Could you check a few things on this model? Use its own coordinates, in mm. A direction names the side the tool comes from. Give positions to 0.01 mm unless a question says otherwise; leave off trailing zeros. Order: outer loops, then holes, each group sorted by start corner. A loop starts at its lowest first (then second) coordinate and runs counter-clockwise, first axis right, second up. Notation, with made-up numbers: M -34,13.5 L 17,13.5 A14 cw 17,26.5 Z; hole C 51.5,-27 d10. An arc over 180 degrees is marked long. Use a Markdown table: item, result. Add a question column.
Item 1: If I drill on L1, parallel to Y at x = 0, z = 54.5; L2, parallel to Y at x = 0, z = 62.5; L3, parallel to Z at x = -3.5, y = 6.25, over which ranges is the centre line in solid material (lowest first)? Write a range as from..to.
Item 2: Suppose I cut it at A-A on y = 0. Write out the boundary of the cut face in (x, z).
Item 3: For faces 1 (the face through (-3, -1, 125)), 2 (the face through (-6, 0, 90)), 3 (the face through (0, 7, 45)), which set-ups out of +Z, -Z, +X, -X, +Y, -Y let a thin tool reach every point of the face, with its end or its side?
Item 4: I'm going to push flat-ended pins straight in: pin 1 Ø5 at (y, z) = (3.5, 19.5) entering from -X; pin 2 Ø8 at (x, z) = (5, 21) entering from -Y; pin 3 Ø2 at (y, z) = (-5.5, 22.5) entering from +X; pin 4 Ø3.5 at (x, y) = (0, 0) entering from -Z. Where does each tip first touch, or does it pass through?
Item 5: Suppose I cut it at C-C on z = 103.5. Write out the boundary of the cut face in (x, y), plus the area to 3 significant figures.
Item 6: Suppose I cut it at D-D on z = 16. Write out the boundary of the cut face in (x, y), plus the area to 3 significant figures.
Item 7: If we mould it in two halves opening along X, with no side actions, what happens to faces 4 (the face through (-5.158, -3.955, 39.93)), 5 (the face through (1, 3, 0)), 6 (the face through (-3, 0, 62))? For each: released by +X, released by -X, zero draft, split by the parting line, or undercut.
from build123d import *

# Parameters (mm, degrees)
SKETCH1_R           = 5
SKETCH1_R_2         = 3
BOSS_EXTRUDE1_DEPTH = 35
SKETCH2_R           = 6.5
SKETCH2_R_2         = 3
BOSS_EXTRUDE2_DEPTH = 10
SKETCH3_R           = 8
SKETCH3_R_2         = 3
BOSS_EXTRUDE3_DEPTH = 10
SKETCH4_R           = 6
SKETCH4_R_2         = 3
BOSS_EXTRUDE4_DEPTH = 70
CHAMFER1_SIZE       = 1
CHAMFER1_SIZE2      = 10


with BuildPart() as part:
    # Sketch1 → Boss-Extrude1 (new body)
    with BuildSketch(Plane.XY):
        Circle(SKETCH1_R)
        Circle(SKETCH1_R_2, mode=Mode.SUBTRACT)
    extrude(amount=BOSS_EXTRUDE1_DEPTH)

    # Sketch2 → Boss-Extrude2 (add)
    with BuildSketch(Plane.XY.offset(35)):
        Circle(SKETCH2_R)
        Circle(SKETCH2_R_2, mode=Mode.SUBTRACT)
    extrude(amount=BOSS_EXTRUDE2_DEPTH)

    # Sketch3 → Boss-Extrude3 (add)
    with BuildSketch(Plane.XY.offset(45)):
        Circle(SKETCH3_R)
        Circle(SKETCH3_R_2, mode=Mode.SUBTRACT)
    extrude(amount=BOSS_EXTRUDE3_DEPTH)

    # Sketch4 → Boss-Extrude4 (add)
    with BuildSketch(Plane.XY.offset(55)):
        Circle(SKETCH4_R)
        Circle(SKETCH4_R_2, mode=Mode.SUBTRACT)
    extrude(amount=BOSS_EXTRUDE4_DEPTH)

    # Chamfer1
    chamfer1_edges = [part.edges().sort_by_distance(p)[0] for p in [
        (-5, 0, 0),
    ]]
    chamfer1_side = [part.faces().sort_by_distance(p)[0] for p in [
        (-4.858578644, 0, 0),
    ]]
    chamfer(chamfer1_edges, length=CHAMFER1_SIZE, length2=CHAMFER1_SIZE2, reference=chamfer1_side[0])


solid = part.part
Findings below:
| question | item | result |
|---|---|---|
| 1 | L1 | y = -8..-3, 3..8 |
| 1 | L2 | y = -6..-3, 3..6 |
| 1 | L3 | z = 45..55 |
| 2 | outline | M -8,45 L -6.5,45 L -6.5,35 L -5,35 L -5,10 L -4,0 L -3,0 L -3,125 L -6,125 L -6,55 L -8,55 Z; M 3,0 L 4,0 L 5,10 L 5,35 L 6.5,35 L 6.5,45 L 8,45 L 8,55 L 6,55 L 6,125 L 3,125 Z |
| 3 | face 1 | +Z, +X, -X, +Y, -Y |
| 3 | face 2 | +Z |
| 3 | face 3 | -Z |
| 4 | pin 1 | stops at x = -4.9 |
| 4 | pin 2 | stops at y = -4.9 |
| 4 | pin 3 | stops at x = 2.18 |
| 4 | pin 4 | passes through |
| 5 | outline | C 0,0 d12; hole C 0,0 d6 |
| 5 | area | 84.8 mm^2 |
| 6 | outline | C 0,0 d10; hole C 0,0 d6 |
| 6 | area | 50.3 mm^2 |
| 7 | face 4 | split by the parting line |
| 7 | face 5 | zero draft |
| 7 | face 6 | undercut |
